Source: CAD feature listing. Evaluate the final solid. Frame: model axes, mm. Face numbers are marked on the shaded views. A direction names the side the tool comes from. Coordinates: 2 decimals unless noted, no trailing zeros. Loops run counter-clockwise (first coordinate to the right, second up) from the corner with the lowest first, then second, coordinate; pieces in that order, holes last.
from build123d import *

# Parameters (mm, degrees)
BOSS_EXTRUDE1_DEPTH = 200
BOSS_EXTRUDE2_DEPTH = 5
CUT_EXTRUDE1_DEPTH  = 5
LPATTERN1_COUNT     = 4
LPATTERN1_PITCH     = 120
SKETCH5_R           = 3
CUT_EXTRUDE2_DEPTH  = 399.319386088
CUT_EXTRUDE4_DEPTH  = 10
CUT_EXTRUDE5_DEPTH  = 10


with BuildPart() as part:
    # Sketch1 → Boss-Extrude1 (new, symmetric)
    with BuildSketch(Plane(origin=(0, 0, 0), x_dir=(1, 0, 0), z_dir=(0, 1, 0))):
        Polygon((0, 17.320508076), (-15, 8.660254038), (-15, -8.660254038), (0, -17.320508076), (15, -8.660254038), (15, 8.660254038), align=None)
        Polygon((-12, 6.92820323), (-12, -6.92820323), (0, -13.856406461), (12, -6.92820323), (12, 6.92820323), (0, 13.856406461), align=None, mode=Mode.SUBTRACT)
    extrude(amount=BOSS_EXTRUDE1_DEPTH, both=True)

    # Sketch2 → Boss-Extrude2 (add)
    with BuildSketch(Plane(origin=(0, 170, 0), x_dir=(1, 0, 0), z_dir=(0, 1, 0))):
        Polygon((0, 46.188021535), (-40, -23.094010768), (40, -23.094010768), align=None)
        Polygon((15, 8.660254038), (0, 17.320508076), (-15, 8.660254038), (-15, -8.660254038), (0, -17.320508076), (15, -8.660254038), align=None, mode=Mode.SUBTRACT)
    boss_extrude2 = extrude(amount=-BOSS_EXTRUDE2_DEPTH)

    # Sketch3 → Cut-Extrude1 (cut)
    with BuildSketch(Plane.XZ.offset(-165)):
        Polygon((0, -46.188021535), (5, -37.527767497), (-5, -37.527767497), align=None)
        Polygon((40, 23.094010768), (30, 23.094010768), (35, 14.43375673), align=None)
        Polygon((-40, 23.094010768), (-35, 14.43375673), (-30, 23.094010768), align=None)
    cut_extrude1 = extrude(amount=-CUT_EXTRUDE1_DEPTH, mode=Mode.SUBTRACT)

    # LPattern1: Boss-Extrude2, Cut-Extrude1 ×4
    with Locations(*[(0, -i * LPATTERN1_PITCH, 0) for i in range(1, LPATTERN1_COUNT)]):
        add(boss_extrude2)
        add(cut_extrude1, mode=Mode.SUBTRACT)

    # Sketch5 → Cut-Extrude2 (cut, through all)
    with BuildSketch(Plane.XZ.offset(195)):
        with Locations(Location((-25, 14.43375673, 0), (0, 0, 270))):
            Circle(SKETCH5_R)
        with Locations(Location((25, 14.43375673, 0), (0, 0, 270))):
            Circle(SKETCH5_R)
        with Locations(Location((0, -28.867513459, 0), (0, 0, 270))):
            Circle(SKETCH5_R)
    extrude(amount=-CUT_EXTRUDE2_DEPTH, mode=Mode.SUBTRACT)

    # Sketch7 → Cut-Extrude4 (cut)
    with BuildSketch(Plane.XZ.offset(-165)):
        Polygon((30, 23.094010768), (-30, 23.094010768), (-35, 14.43375673), (-5, -37.527767497), (5, -37.527767497), (35, 14.43375673), align=None)
        Polygon((-15, -8.660254038), (-15, 8.660254038), (0, 17.320508076), (15, 8.660254038), (15, -8.660254038), (0, -17.320508076), align=None, mode=Mode.SUBTRACT)
    extrude(amount=-CUT_EXTRUDE4_DEPTH, mode=Mode.SUBTRACT)

    # Sketch8 → Cut-Extrude5 (cut)
    with BuildSketch(Plane.XZ.offset(75)):
        Polygon((-35, 14.43375673), (-5, -37.527767497), (5, -37.527767497), (35, 14.43375673), (30, 23.094010768), (-30, 23.094010768), align=None)
        Polygon((0, 17.320508076), (15, 8.660254038), (15, -8.660254038), (0, -17.320508076), (-15, -8.660254038), (-15, 8.660254038), align=None, mode=Mode.SUBTRACT)
    extrude(amount=-CUT_EXTRUDE5_DEPTH, mode=Mode.SUBTRACT)


solid = part.part
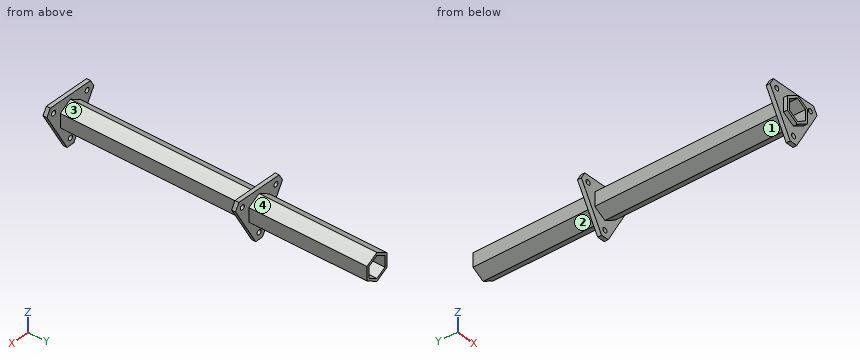
Q1. Contact query for flat-ended pins moving along their axis: pin 1 Ø8 at (x, z) = (-25, 14.43) entering from +Y; pin 2 Ø14 at (y, z) = (-130.5, -1.5) entering from -X; pin 3 Ø5 at (x, y) = (-5.5, -87) entering from -Z; pin 4 Ø3 at (x, z) = (-10, 0.5) entering from +Y. Output: stop coordinate, or through.
Q2. Draft query along Y for the marked faces 3 and 4. Return one class per face: +Y half, -Y half, draft (parallel to the pull), parting line (faces both ways), or undercut.
Q3. Line query: line 1 along X through (y, z) = (24, -5.5); line 2 along Y through (x, z) = (15, 13.5); line 3 along Z through (x, y) = (0, -112). Output: solid intervals per line, ascending.
Q4. Section A-A, the plane y = -172. Return the cut outline in (x, z).
Q5. Access query for the marked faces 1 and 2. Directions: +Z, -Z, +X, -X, +Y, -Y. A direction counts if a zero-diameter tool reaches every point of the face in a straight line with its end or side. Return the directions, or none.
Derived:
1. pin 1: stops at y = 50
1. pin 2: stops at x = -15
1. pin 3: stops at z = -15.59
1. pin 4: passes through
2. face 3: undercut
2. face 4: draft
3. line 1: x = -15 to -12, 12 to 15
3. line 2: y = -195 to -190, 45 to 50
3. line 3: z = -17.32 to -13.86, 13.86 to 17.32
4. outline: (-15, -8.66) - (0, -17.32) - (15, -8.66) - (15, 8.66) - (0, 17.32) - (-15, 8.66) - close; hole (-12, -6.93) - (0, -13.86) - (12, -6.93) - (12, 6.93) - (0, 13.86) - (-12, 6.93) - close
5. face 1: -Z, -X
5. face 2: -Z, -X, +Y
